```python
from build123d import *

# Parameters (mm, degrees)
BASE_BLOCK_PROFILE_W       = 63
BASE_BLOCK_PROFILE_H       = 30
BASE_BLOCK_DEPTH           = 26
STEPPED_SLOPE_CUT_DEPTH    = 26
INCLINED_CHANNEL_CUT_DEPTH = 44
CENTRE_RIB_PROFILE_W       = 8
CENTRE_RIB_PROFILE_H       = 25.036205804
CENTRE_RIB_DEPTH           = 30
TOP_NOTCH_CUT_DEPTH        = 30


with BuildPart() as part:
    # Base Block Profile → Base Block (new body)
    with BuildSketch(Plane(origin=(0, 0, 0), x_dir=(0, 0, -1), z_dir=(1, 0, 0))):
        Rectangle(BASE_BLOCK_PROFILE_W, BASE_BLOCK_PROFILE_H)
    extrude(amount=BASE_BLOCK_DEPTH)

    # Stepped Slope Profile → Stepped Slope Cut (cut)
    with BuildSketch(Plane(origin=(26, 0, 0), x_dir=(0, 0, -1), z_dir=(1, 0, 0))):
        Polygon((-31.5, 15), (-31.5, -2), (-21.5, -2), (0, 10), (0, 15), align=None)
    extrude(amount=-STEPPED_SLOPE_CUT_DEPTH, mode=Mode.SUBTRACT)

    # Inclined Channel Profile → Inclined Channel Cut (cut)
    with BuildSketch(Plane(origin=(0, 15, 0), x_dir=(1, 0, 0), z_dir=(0, 1, 0))):
        Polygon((8.908390329, 0), (5, 0), (5, -21.5), (21, -21.5), (21, 0), (16.908390329, 0), (16.908390329, -13.5), (8.908390329, -13.5), align=None)
    extrude(amount=-INCLINED_CHANNEL_CUT_DEPTH, mode=Mode.SUBTRACT)

    # Centre Rib Profile → Centre Rib (add)
    with BuildSketch(Plane.XZ.offset(15)):
        with Locations((12.908390329, 0.981897098)):
            Rectangle(CENTRE_RIB_PROFILE_W, CENTRE_RIB_PROFILE_H)
    extrude(amount=-CENTRE_RIB_DEPTH)

    # Notch Profile → Top Notch Cut (cut)
    with BuildSketch(Plane(origin=(16.908390329, 0, 0), x_dir=(0, 0, -1), z_dir=(1, 0, 0))):
        Polygon((0, 10), (-13.5, 2.465116279), (-13.5, 15), (0, 15), align=None)
    extrude(amount=-TOP_NOTCH_CUT_DEPTH, mode=Mode.SUBTRACT)


solid = part.part
```
Build history of the part. All positions in model axes, mm. A direction names the side the tool comes from. Give positions to 0.01 mm unless a question says otherwise; leave off trailing zeros. Loops run counter-clockwise (first coordinate to the right, second up) from the corner with the lowest first, then second, coordinate; pieces in that order, holes last. Notation, with made-up numbers: (78.25, 75.5) - (126.25, 75.5) arc R20 ccw to (126.25, 87.5) - close; hole circle Ø4 at (7.5, 56.25). An arc over 180 degrees is marked (long way). Use a Markdown table: item, result.
(1) Drop flat-ended pins along their axis: pin 1 Ø2 at (x, y) = (15.5, 9.5) entering from +Z; pin 2 Ø8 at (x, z) = (22, 8.5) entering from +Y; pin 3 Ø5 at (x, z) = (19, 28) entering from +Y. Give the stop position or say it passes through.
Taken from the geometry:
| item | result |
|---|---|
| pin 1 | z = 2.69 |
| pin 2 | y = 7.49 |
| pin 3 | y = -2 |
(2) Band-saw the part on D-D (y = 6.5). Give the cut face in (x, z).
Taken from the geometry:
| item | result |
|---|---|
| outline | (0, -31.5) - (26, -31.5) - (26, 6.27) - (21, 6.27) - (21, 0) - (16.91, 0) - (16.91, 6.27) - (8.91, 6.27) - (8.91, 0) - (5, 0) - (5, 6.27) - (0, 6.27) - close |
(3) Which spindle directions (+Z, -Z, +X, -X, +Y, -Y) get a long thin tool onto all of the face, cutting with end or side? Do faces 1 (the face through (8.908, -5, 7)), 2 (the face through (13, -2, 27)), 3 (the face through (13, -15, 0)). Say none if no direction does.
Taken from the geometry:
| item | result |
|---|---|
| face 1 | +Y, -Y |
| face 2 | +Z, +X, -X, +Y |
| face 3 | +Z, -Z, +X, -X, -Y |
(4) Wall check: line 1 along X through (y, z) = (4.5, 5); line 2 along Z through (x, y) = (10, -10.5); line 3 along Z through (x, y) = (20.5, -7.5). Give the ranges that are in metal, low to high.
Taken from the geometry:
| item | result |
|---|---|
| line 1 | 0 to 5, 8.91 to 16.91, 21 to 26 |
| line 2 | -31.5 to 13.5, 21.5 to 31.5 |
| line 3 | -31.5 to 0, 21.5 to 31.5 |
(5) Pull direction X, two halves, no side cores. Call faces 4 (the face through (18, 4, 0)), 5 (the face through (26, -3, -7)), 6 (the face through (13, 0, -31.5)), 7 (the face through (0, -3, -7)): +X half, -X half, draft (parallel to the pull), parting line (faces both ways), or undercut.
Taken from the geometry:
| item | result |
|---|---|
| face 4 | undercut |
| face 5 | +X half |
| face 6 | draft |
| face 7 | -X half |
(6) Band-saw the part on C-C (z = 11). Give the cut face in (x, y).
Taken from the geometry:
| item | result |
|---|---|
| outline | (0, -15) - (5, -15) - (5, 3.86) - (0, 3.86) - close; (8.91, -15) - (16.91, -15) - (16.91, 3.86) - (8.91, 3.86) - close; (21, -15) - (26, -15) - (26, 3.86) - (21, 3.86) - close |
(7) Band-saw the part on A-A (y = -4.75). Give the cut face in (x, z).
Taken from the geometry:
| item | result |
|---|---|
| outline | (0, -31.5) - (26, -31.5) - (26, 31.5) - (0, 31.5) - close; hole (5, 0) - (8.91, 0) - (8.91, 13.5) - (16.91, 13.5) - (16.91, 0) - (21, 0) - (21, 21.5) - (5, 21.5) - close |
(8) Band-saw the part on B-B (x = 15.5). Give the cut face in (y, z).
Taken from the geometry:
| item | result |
|---|---|
| outline | (-15, -31.5) - (15, -31.5) - (15, 0) - (10, 0) - (2.47, 13.5) - (-15, 13.5) - close; (-15, 21.5) - (-2, 21.5) - (-2, 31.5) - (-15, 31.5) - close |
